For this review, take the finished solid that the model builds, in its own axes (mm). A direction names the side the tool comes from. Round coordinates to 2 decimals unless told otherwise and drop trailing zeros. Write each loop counter-clockwise with the first axis right and the second up, starting at its lowest first coordinate (ties: lowest second). Pieces come first, ordered by that corner, then holes. Notation, with made-up numbers: (-13, 23) - (30, 23) arc R11 ccw to (30, 43) - close; hole circle Ø4 at (76, -15.5). An arc over 180 degrees is marked (long way). One line per item, written item: value. Start each with the question number.
Q1. Mouldability with a two-part tool opening along X and no side actions: class faces 5 (the face through (212, 1233.6, -75)), 6 (the face through (220.09, 706.84, -79.84)), 7 (the face through (254.5, 709, -75)), 8 (the face through (230.75, 1032.37, -51.19)) as +X half, -X half, draft (parallel to the pull), parting line (faces both ways), or undercut.
Q2. For probe 1 along Y at (x, z) = (189.5, -78); probe 2 along Y at (x, z) = (222, -59); probe 3 along Z at (x, y) = (212, 1016), list the stretches that pass through material, from the lowest coordinate up.
Q3. Clearance check with flat-ended pins moving along their axes: pin 1 Ø2 at (x, z) = (255.5, -69) entering from -Y; pin 2 Ø4 at (x, y) = (219, 991.5) entering from +Z; pin 3 Ø5 at (x, z) = (226, -56.5) entering from -Y; pin 4 Ø13.5 at (x, y) = (234.5, 700.5) entering from -Z. State where each tip first meets the part, or that it passes through.
Q4. Add section B-B on y = 795.5. Write out the cut boundary in (x, z).
Q5. Tool access review of faces 1 (the face through (237, 732, -90)), 2 (the face through (188, 1215.6, -59)), 3 (the face through (237, 732, -60)), 4 (the face through (230.75, 1192.81, -51.19)): name each direction out of +Z, -Z, +X, -X, +Y, -Y from which nothing blocks a thin tool from reaching the whole face with its end or side.
Q6. Add section A-A on y = 972. Write out the cut boundary in (x, z).
```python
from build123d import *

# Parameters (mm, degrees)
SKETCH_2_R           = 24
SHELL_1_T            = -5
SKETCH_4_R           = 60
EXTRUDE_1_DEPTH      = 6
SKETCH_5_W           = 200
SKETCH_5_H           = 250
EXTRUDE_2_DEPTH      = 280
SKETCH_6_R           = 30
EXTRUDE_3_DEPTH      = 97.1
SKETCH_7_R           = 29.5
EXTRUDE_4_DEPTH      = 5
SKETCH_8_R           = 30
EXTRUDE_5_DEPTH      = 35
SKETCH_9_R           = 29.5
EXTRUDE_6_DEPTH      = 5
SKETCH_10_R          = 30
EXTRUDE_7_DEPTH      = 41
SKETCH_11_R          = 29.5
EXTRUDE_8_DEPTH      = 5
SKETCH_12_R          = 30
EXTRUDE_9_DEPTH      = 41
SKETCH_13_R          = 29
EXTRUDE_10_DEPTH     = 2
SKETCH_14_R          = 30
EXTRUDE_11_DEPTH     = 18
FILLET_1_R           = 3
SKETCH_15_OUTSIDE_W  = 599.076
SKETCH_15_OUTSIDE_H  = 512.576
SKETCH_15_OUTSIDE_R  = 22.5
CUT_EXTRUDE_1_DEPTH  = 26
SKETCH_16_W          = 1000.950512006
SKETCH_16_H          = 1372.546192884
CUT_EXTRUDE_12_DEPTH = 1285.766986682
SKETCH_17_R          = 12.5
EXTRUDE_13_DEPTH     = 27
SKETCH_24_R          = 9
EXTRUDE_1_2_DEPTH    = 275
EXTRUDE_1_3_DEPTH    = 15


with BuildPart() as part:
    # 扫描4: sweep along a path in 草图1
    with BuildLine(Plane.XY) as sweep_4_path:
        Line((0, 0), (0, 202.5))
        ThreePointArc((0, 202.5), (8.786796564, 223.713203436), (30, 232.5))
        Line((30, 232.5), (182.5, 232.5))
        ThreePointArc((182.5, 232.5), (203.713203436, 241.286796564), (212.5, 262.5))
        Line((212.5, 262.5), (212.5, 698.5))
    # 草图2 → 扫描4 (sweep)
    with BuildSketch(Plane(origin=(0, 0, 0), x_dir=(1, 0, 0), z_dir=(0, 1, 0))):
        Circle(SKETCH_2_R)
    sweep(path=sweep_4_path.line)

    # 抽壳1
    shell_1_openings = [part.faces().sort_by_distance(p)[0] for p in [
        (0, 0, 0),
    ]]
    offset(amount=SHELL_1_T, openings=shell_1_openings, kind=Kind.INTERSECTION)

    # 草图4 → Extrude 1 (add)
    with BuildSketch(Plane(origin=(0, 698.5, 0), x_dir=(-1, 0, 0), z_dir=(0, 1, 0))):
        with Locations(Location((-212.5, 0, 0), (0, 0, 90))):
            Circle(SKETCH_4_R)
    extrude(amount=EXTRUDE_1_DEPTH)

    # 草图5 → 拉伸2 (add)
    with BuildSketch(Plane(origin=(0, 704.5, 0), x_dir=(-1, 0, 0), z_dir=(0, 1, 0))):
        with Locations((-212.5, 0)):
            Rectangle(SKETCH_5_W, SKETCH_5_H)
    extrude(amount=EXTRUDE_2_DEPTH)

    # 草图6 → 拉伸3 (add)
    with BuildSketch(Plane(origin=(0, 984.5, 0), x_dir=(-1, 0, 0), z_dir=(0, 1, 0))):
        with Locations(Location((-212.5, -75, 0), (0, 0, 270))):
            Circle(SKETCH_6_R)
    extrude(amount=EXTRUDE_3_DEPTH)

    # 草图7 → 拉伸4 (add)
    with BuildSketch(Plane(origin=(0, 1081.6, 0), x_dir=(-1, 0, 0), z_dir=(0, 1, 0))):
        with Locations(Location((-212.5, -75, 0), (0, 0, 90))):
            Circle(SKETCH_7_R)
    extrude(amount=EXTRUDE_4_DEPTH)

    # 草图8 → 拉伸5 (add)
    with BuildSketch(Plane(origin=(0, 1086.6, 0), x_dir=(-1, 0, 0), z_dir=(0, 1, 0))):
        with Locations(Location((-212.5, -75, 0), (0, 0, 270))):
            Circle(SKETCH_8_R)
    extrude(amount=EXTRUDE_5_DEPTH)

    # 草图9 → 拉伸6 (add)
    with BuildSketch(Plane(origin=(0, 1121.6, 0), x_dir=(-1, 0, 0), z_dir=(0, 1, 0))):
        with Locations(Location((-212.5, -75, 0), (0, 0, 90))):
            Circle(SKETCH_9_R)
    extrude(amount=EXTRUDE_6_DEPTH)

    # 草图10 → 拉伸7 (add)
    with BuildSketch(Plane(origin=(0, 1126.6, 0), x_dir=(-1, 0, 0), z_dir=(0, 1, 0))):
        with Locations(Location((-212.5, -75, 0), (0, 0, 270))):
            Circle(SKETCH_10_R)
    extrude(amount=EXTRUDE_7_DEPTH)

    # 草图11 → 拉伸8 (add)
    with BuildSketch(Plane(origin=(0, 1167.6, 0), x_dir=(-1, 0, 0), z_dir=(0, 1, 0))):
        with Locations(Location((-212.5, -75, 0), (0, 0, 90))):
            Circle(SKETCH_11_R)
    extrude(amount=EXTRUDE_8_DEPTH)

    # 草图12 → 拉伸9 (add)
    with BuildSketch(Plane(origin=(0, 1172.6, 0), x_dir=(-1, 0, 0), z_dir=(0, 1, 0))):
        with Locations(Location((-212.5, -75, 0), (0, 0, 270))):
            Circle(SKETCH_12_R)
    extrude(amount=EXTRUDE_9_DEPTH)

    # 草图13 → 拉伸10 (add)
    with BuildSketch(Plane(origin=(0, 1213.6, 0), x_dir=(-1, 0, 0), z_dir=(0, 1, 0))):
        with Locations(Location((-212.5, -75, 0), (0, 0, 90))):
            Circle(SKETCH_13_R)
    extrude(amount=EXTRUDE_10_DEPTH)

    # 草图14 → 拉伸11 (add)
    with BuildSketch(Plane(origin=(0, 1215.6, 0), x_dir=(-1, 0, 0), z_dir=(0, 1, 0))):
        with Locations(Location((-212.5, -75, 0), (0, 0, 270))):
            Circle(SKETCH_14_R)
    extrude(amount=EXTRUDE_11_DEPTH)

    # 圆角1
    fillet_1_edges = [part.edges().sort_by_distance(p)[0] for p in [
        (212.5, 1233.6, -45),
    ]]
    fillet(fillet_1_edges, radius=FILLET_1_R)

    # 草图15 outside → 切除-拉伸1 (cut)
    with BuildSketch(Plane.XZ):
        with Locations((144.25, 0)):
            Rectangle(SKETCH_15_OUTSIDE_W, SKETCH_15_OUTSIDE_H)
        with Locations(Location((0, 0, 0), (0, 0, 270))):
            Circle(SKETCH_15_OUTSIDE_R, mode=Mode.SUBTRACT)
    extrude(amount=-CUT_EXTRUDE_1_DEPTH, mode=Mode.SUBTRACT)

    # 草图16 → 拉伸12 (cut, through all)
    with BuildSketch(Plane(origin=(312.5, 0, 0), x_dir=(0, 0, -1), z_dir=(1, 0, 0))):
        with Locations((-375.475256003, 298.226903558)):
            Rectangle(SKETCH_16_W, SKETCH_16_H)
    extrude(amount=-CUT_EXTRUDE_12_DEPTH, mode=Mode.SUBTRACT)

    # 草图17 → 拉伸13 (add)
    with BuildSketch(Plane.XZ.offset(-984.5)):
        with Locations(Location((212.5, -75, 0), (0, 0, 90))):
            Circle(SKETCH_17_R)
    extrude(amount=EXTRUDE_13_DEPTH)

    # 草图24 → Extrude 1 2 (add)
    with BuildSketch(Plane.XZ.offset(-957.5)):
        with Locations(Location((212.5, -75, 0), (0, 0, 270))):
            Circle(SKETCH_24_R)
    extrude(amount=EXTRUDE_1_2_DEPTH)

    # 草图26 → Extrude 1 3 (add, symmetric)
    with BuildSketch(Plane.XY.offset(-75)):
        Polygon((186.5, 732.5), (256.5, 732.5), (256.5, 687.5), (254.5, 687.5), (254.5, 730.5), (186.5, 730.5), align=None)
    extrude(amount=EXTRUDE_1_3_DEPTH, both=True)


solid = part.part
```
Result set:
1. face 5: draft
1. face 6: undercut
1. face 7: undercut
1. face 8: parting line
2. probe 1: y = 730.5 to 732.5, 984.5 to 1233.6
2. probe 2: y = 984.5 to 1233.6
2. probe 3: z = -105 to -45
3. pin 1: stops at y = 687.5
3. pin 2: stops at z = -45.34
3. pin 3: stops at y = 984.5
3. pin 4: passes through
4. outline: circle Ø18 at (212.5, -75)
5. face 1: -Z, +X, -X, -Y
5. face 2: none
5. face 3: +Z, +X, -X, -Y
5. face 4: +Y
6. outline: circle Ø25 at (212.5, -75)
